Part print with two shaded views. Sizes in mm from the minimum x, y, z corner. A direction names the side the tool comes from. Coordinates: 2 decimals unless noted, no trailing zeros. Write each loop counter-clockwise with the first axis right and the second up, starting at its lowest first coordinate (ties: lowest second). Pieces come first, ordered by that corner, then holes.
Q1. Pin check, flat tips, straight feed: P1, Ø1, axis at x = 15.5, y = 6, coming from the +Z side; P2, Ø1.5, axis at y = 17.5, z = 88, coming from the -X side; P3, Ø5, axis at x = 56.5, y = 28.5, coming from the +Z side; P4, Ø10, axis at x = 47, z = 61, coming from the -Y side. Stop position of each tip, or through.
Q2. Band-saw the part on D-D, the plane z = 30. Write the cut outline in (x, y), plus the area to 3 significant figures.
Q3. Band-saw the part on B-B, the plane z = 65. Write the cut outline in (x, y), plus the area to 3 significant figures.
Q4. Band-saw the part on A-A, the plane x = 65. Write the cut outline in (y, z), plus the area to 3 significant figures.
Q5. Drill centre lines: probe 1 along X at (y, z) = (31, 65); probe 2 along X at (y, z) = (12.5, 65); probe 3 along Y at (x, z) = (91, 33). Where is each one in solid material? Low to high.
Q6. Which spindle directions (+Z, -Z, +X, -X, +Y, -Y) get a long thin tool onto all of the face, cutting with end or side? Do the marked faces 1 and 2. Say none if no direction does.
Q7. Pull direction X, two halves, no side cores. Call the marked faces 3, 4 and 5: released by +X, released by -X, zero draft, split by the parting line, or undercut.
Q8. Band-saw the part on C-C, the plane y = 33. Write the cut outline in (x, z), plus the area to 3 significant figures.
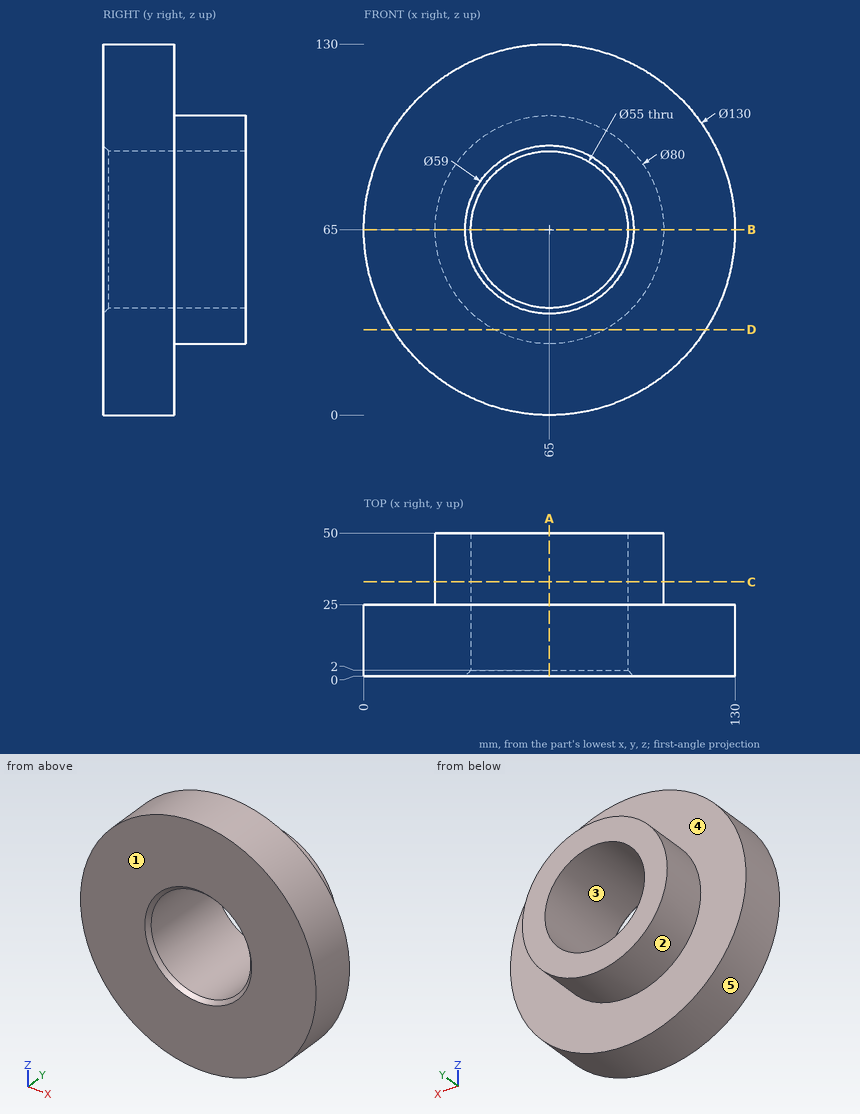
Answer sheet:
1. P1: stops at z = 107.71
1. P2: stops at x = 3.93
1. P3: stops at z = 104.55
1. P4: passes through
2. outline: (10.23, 0) - (119.77, 0) - (119.77, 25) - (84.36, 25) - (84.36, 50) - (45.64, 50) - (45.64, 25) - (10.23, 25) - close
2. area: 3,710 mm2
3. outline: (0, 0) - (35.5, 0) - (37.5, 2) - (37.5, 50) - (25, 50) - (25, 25) - (0, 25) - close; (92.5, 2) - (94.5, 0) - (130, 0) - (130, 25) - (105, 25) - (105, 50) - (92.5, 50) - close
3. area: 2,500 mm2
4. outline: (0, 0) - (25, 0) - (25, 25) - (50, 25) - (50, 37.5) - (2, 37.5) - (0, 35.5) - close; (0, 94.5) - (2, 92.5) - (50, 92.5) - (50, 105) - (25, 105) - (25, 130) - (0, 130) - close
4. area: 2,500 mm2
5. probe 1: x = 25 to 37.5, 92.5 to 105
5. probe 2: x = 0 to 37.5, 92.5 to 130
5. probe 3: y = 0 to 25
6. face 1: +Z, -Z, +X, -X, -Y
6. face 2: +Y
7. face 3: undercut
7. face 4: zero draft
7. face 5: split by the parting line
8. outline: circle Ø80 at (65, 65); hole circle Ø55 at (65, 65)
8. area: 2,650 mm2
